Geometry: see drawing. Coordinates: mm, zero at the bounding-box minimum. Give positions to 0.01 mm unless a question says otherwise; leave off trailing zeros. Loops run counter-clockwise (first coordinate to the right, second up) from the corner with the lowest first, then second, coordinate; pieces in that order, holes last. Notation, with made-up numbers: (18, 64.5) -> (51, 64.5) arc R26 cw to (51, 87.5) -> close; hole circle Ø2 at (39, -36). An arc over 180 degrees is marked (long way). Return JSON: item names as keys, results as strings. Group by question number.
(1) Cut plane B-B on y = 153. Return loops of the section in (x, z), then the cut area to 3 significant figures.
(2) Cut plane A-A on z = 4.25. Return loops of the section in (x, y).
(3) Cut plane C-C on x = 85.5. Return loops of the section in (y, z), then the cut area to 3 significant figures.
(4) Ray query, line 1 (Y direction, x = 75, z = 8.5); line 2 (X direction, y = 124.5, z = 3.5); line 3 (X direction, y = 48, z = 2). Return the intervals inside material, ascending. Write a range as from..to.
(5) Pin query (flat end, axial travel): pin 1 (1 mm diameter, centred on y = 71.5, z = 8.5, fed in from +X); pin 2 (3 mm diameter, centred on y = 152.5, z = 1.5, fed in from +X). Return the tip coordinate at first contact, or that it passes through.
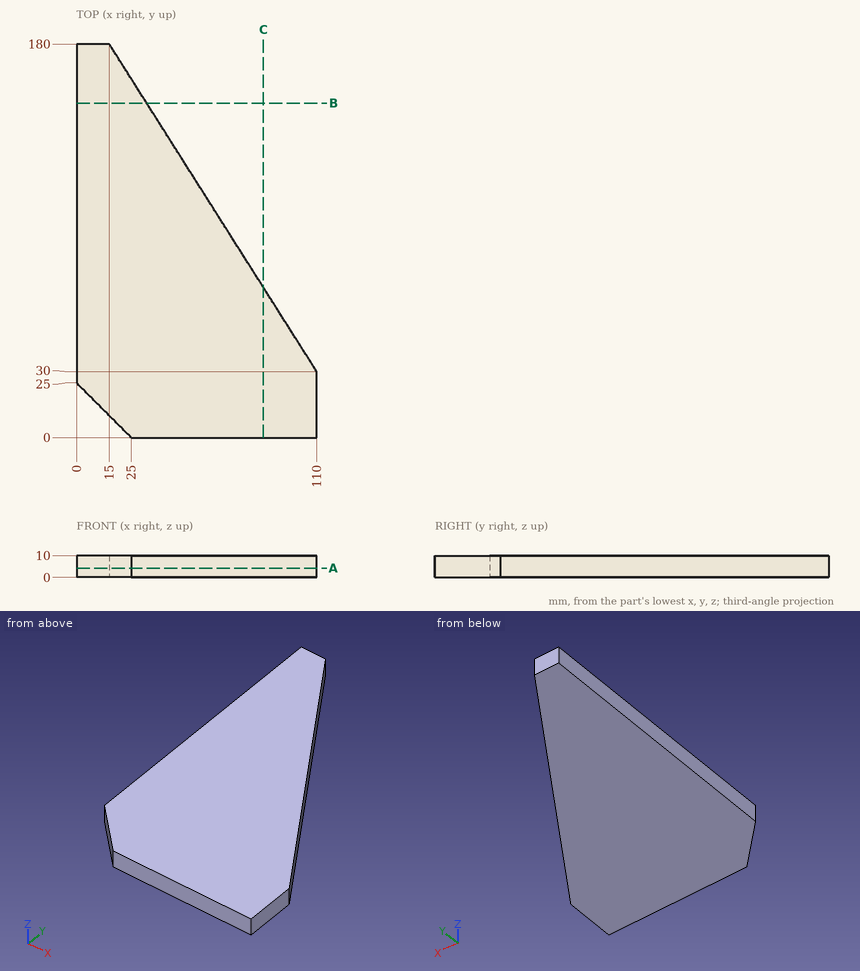
Answers:
{
 "1": {"outline": "(0, 0) -> (32.1, 0) -> (32.1, 10) -> (0, 10) -> close", "area": "321 mm²"},
 "2": {"outline": "(0, 25) -> (25, 0) -> (110, 0) -> (110, 30) -> (15, 180) -> (0, 180) -> close"},
 "3": {"outline": "(0, 0) -> (68.68, 0) -> (68.68, 10) -> (0, 10) -> close", "area": "687 mm²"},
 "4": {"line 1": "0..85.26", "line 2": "0..50.15", "line 3": "0..98.6"},
 "5": {"pin 1": "x = 84.03", "pin 2": "x = 33.37"}
}
